Can you work these out from the model? Positions are in its coordinate system, mm. A direction names the side the tool comes from. Coordinates: 2 decimals unless noted, no trailing zeros. Order: outer loops, then holes, each group sorted by start corner. A loop starts at its lowest first (then second) coordinate and runs counter-clockwise, first axis right, second up. Notation, with made-up numbers: (14, -37) - (30, -37) arc R8 cw to (30, -26) - close; hole circle Ø1 at (86, -27). An arc over 180 degrees is marked (long way). Use a Markdown table: item, result. Add a question column.
(1) I want a section at A-A (z = 125). List the corners of the cut face in (x, y) for me, and give its area (3 significant figures).
(2) If I drill on L1, parallel to X at y = -0.75, z = 113.5; L2, parallel to X at y = 2.25, z = 64; L3, parallel to Z at x = 5.75, y = -2.5, over which ranges is the centre line in solid material (lowest first)? Write a range as [from, to].
(3) On a 3-axis mill with a long thin cutter (end or side, diameter ignored), from which of +Z, -Z, +X, -X, +Y, -Y can I reach the whole of each face in a straight line? I mean faces 1 (the cylindrical face through (-11, 0, 53)), 2 (the cylindrical face through (5, 1.6, 50.4)), 3 (the cylindrical face through (-0.07, 1.73, 117.19)), 4 (the flat face through (-5, 0, 114)), 5 (the flat face through (5, 0, 114)). Say none if no direction works.
(4) We'd pull the mould along Y, two halves only. Please class faces 6 (the conical face through (-0.87, 0.274, 102.107)), 7 (the flat face through (4, -4, 0)), 8 (the cylindrical face through (-0.07, -0.174, 139.865)): pulls with the +Y half, pulls with the -Y half, needs draft (parallel to the pull), parting line crosses it, or undercut.
(5) For pin 1 Ø1.5 at (y, z) = (3.5, 66) entering from +X; pin 2 Ø5 at (x, y) = (5.5, -2.5) entering from -Z; pin 3 Ø2 at (x, z) = (-3.5, 121) entering from -Y; pin 4 Ø9.5 at (y, z) = (0, 125) entering from +X, each with a flat end and sliding along its axis, tell me the tip position at first contact or that it passes through.
(6) I want a section at B-B (z = 53). List the corners of the cut face in (x, y) for me.
(7) I want a section at C-C (z = 107.5). List the corners of the cut face in (x, y) for me.
```python
from build123d import *

# Parameters (mm, degrees)
SKETCH1_R                  = 11
BOSS_EXTRUDE1_DEPTH        = 140
CUT_EXTRUDE1_DEPTH         = 141.861634237
CUT_EXTRUDE1_DEPTH_BACK    = 35
SKETCH2_W                  = 16.868879615
SKETCH2_H                  = 32.554880476
SKETCH2_W_2                = 13.301543069
SKETCH2_H_2                = 32.07054439
M12X1_5_TAPPED_HOLE1_D     = 10.5
M12X1_5_TAPPED_HOLE1_DEPTH = 99.5
M12X1_5_TAPPED_HOLE1_TIP   = 3.15451825
CHAMFER1_SIZE              = 1
SKETCH5_R                  = 8
CUT_EXTRUDE2_DEPTH         = 142.340015565


with BuildPart() as part:
    # Sketch1 → Boss-Extrude1 (new body)
    with BuildSketch(Plane.XY):
        Circle(SKETCH1_R)
    extrude(amount=BOSS_EXTRUDE1_DEPTH)

    # Sketch2 → Cut-Extrude1 (cut, two sides: drawn at the far end of the back side and taken through both)
    with BuildSketch(Plane.XY.offset(140).offset(-CUT_EXTRUDE1_DEPTH_BACK)):
        with Locations((13.434439808, -1.928606663)):
            Rectangle(SKETCH2_W, SKETCH2_H)
        with Locations((-11.650771535, -1.34790253)):
            Rectangle(SKETCH2_W_2, SKETCH2_H_2)
    extrude(amount=CUT_EXTRUDE1_DEPTH + CUT_EXTRUDE1_DEPTH_BACK, mode=Mode.SUBTRACT)

    # M12x1.5 Tapped Hole1
    with Locations(Plane(origin=(-0.000266702, -0.000350185, 0), x_dir=(-1, 0, 0), z_dir=(0, 0, -1))):
        with Locations((0, 0)):
            Hole(M12X1_5_TAPPED_HOLE1_D / 2, depth=M12X1_5_TAPPED_HOLE1_DEPTH)
            with Locations((0, 0, -(M12X1_5_TAPPED_HOLE1_DEPTH + M12X1_5_TAPPED_HOLE1_TIP / 2))):  # 118° drill point
                Cone(0, M12X1_5_TAPPED_HOLE1_D / 2, M12X1_5_TAPPED_HOLE1_TIP, mode=Mode.SUBTRACT)

    # Chamfer1
    chamfer1_edges = [part.edges().sort_by_distance(p)[0] for p in [
        (-11, 0, 0),
    ]]
    chamfer(chamfer1_edges, length=CHAMFER1_SIZE)

    # Sketch5 → Cut-Extrude2 (cut, through all)
    with BuildSketch(Plane.ZY.offset(5)):
        with Locations(Location((125, 0, 0), (0, 0, 270))):
            Circle(SKETCH5_R)
        with BuildLine():
            Line((125, 14.866485564), (182.888016926, 36.743525749))
            Line((182.888016926, 36.743525749), (236.673487902, -7.349157171))
            Line((236.673487902, -7.349157171), (192.77085965, -51.061730756))
            Line((192.77085965, -51.061730756), (125, -14.866485564))
            ThreePointArc((125, -14.866485564), (139.866485564, 0), (125, 14.866485564))
        make_face()
    extrude(amount=-CUT_EXTRUDE2_DEPTH, mode=Mode.SUBTRACT)


solid = part.part
```
Answers follow:
| question | item | result |
|---|---|---|
| 1 | outline | (-5, -9.8) arc R11 ccw to (5, -9.8) - (5, -8) - (-5, -8) - close; (-5, 8) - (5, 8) - (5, 9.8) arc R11 ccw to (-5, 9.8) - close |
| 1 | area | 52.2 mm² |
| 2 | L1 | x = [-5, 5] |
| 2 | L2 | x = [-10.77, -4.74], [4.74, 10.77] |
| 2 | L3 | z = [0, 105] |
| 3 | face 1 | +Z, -Z |
| 3 | face 2 | -Z |
| 3 | face 3 | +X, -X |
| 3 | face 4 | +Z, -X, +Y, -Y |
| 3 | face 5 | +Z, +X, +Y, -Y |
| 4 | face 6 | undercut |
| 4 | face 7 | needs draft |
| 4 | face 8 | parting line crosses it |
| 5 | pin 1 | stops at x = 10.65 |
| 5 | pin 2 | stops at z = 0 |
| 5 | pin 3 | stops at y = -10.71 |
| 5 | pin 4 | passes through |
| 6 | outline | circle Ø22 at (0, 0); hole circle Ø10.5 at (0, 0) |
| 7 | outline | (-5, -9.8) arc R11 ccw to (5, -9.8) - (5, 9.8) arc R11 ccw to (-5, 9.8) - close |
